from build123d import *

# Parameters (mm, degrees)
SKETCH1_W           = 127
SKETCH1_H           = 38.1
SKETCH1_R           = 15
BOSS_EXTRUDE1_DEPTH = 21
BOSS_EXTRUDE2_DEPTH = 6.35
SKETCH4_R           = 1.4
CUT_EXTRUDE2_DEPTH  = 6.35
CUT_EXTRUDE6_DEPTH  = 14.65
CUT_EXTRUDE7_DEPTH  = 73.600774789
SKETCH7_R           = 2.6035
CUT_EXTRUDE8_DEPTH  = 22.86
SKETCH8_W           = 31.75
SKETCH8_H           = 15.875
SKETCH8_R           = 2.6035
BOSS_EXTRUDE3_DEPTH = 9.652
CHAMFER1_SIZE       = 6.35
BOSS_EXTRUDE4_START = -9.652
SKETCH9_W           = 26.681402361
SKETCH9_H           = 11.886393241
SKETCH9_R           = 2.6035
SKETCH9_W_2         = 26.993648234
BOSS_EXTRUDE4_DEPTH = 9.652


with BuildPart() as part:
    # Sketch1 → Boss-Extrude1 (new body)
    with BuildSketch(Plane.XY):
        Rectangle(SKETCH1_W, SKETCH1_H)
        Circle(SKETCH1_R, mode=Mode.SUBTRACT)
    extrude(amount=-BOSS_EXTRUDE1_DEPTH)

    # Sketch3 → Boss-Extrude2 (add)
    with BuildSketch(Plane(origin=(0, 0, -21), x_dir=(-1, 0, 0), z_dir=(0, 0, -1))):
        with BuildLine():
            Line((12.743745366, -19.05), (-12.743745366, -19.05))
            ThreePointArc((-12.743745366, -19.05), (-9.084403439, -28.194328353), (1.02e-07, -32))
            ThreePointArc((1.02e-07, -32), (9.08440351, -28.194328281), (12.743745366, -19.05))
        make_face()
    boss_extrude2 = extrude(amount=-BOSS_EXTRUDE2_DEPTH)

    # Sketch4 → Cut-Extrude2 (cut)
    with BuildSketch(Plane.XY.offset(-14.65)):
        with Locations((0, -27)):
            Circle(SKETCH4_R)
    cut_extrude2 = extrude(amount=-CUT_EXTRUDE2_DEPTH, mode=Mode.SUBTRACT)

    # Mirror1: Boss-Extrude2, Cut-Extrude2 across plane
    add(boss_extrude2.mirror(Plane.ZX))
    add(cut_extrude2.mirror(Plane.ZX), mode=Mode.SUBTRACT)

    # Sketch5 → Cut-Extrude6 (cut)
    with BuildSketch(Plane.XY):
        with BuildLine():
            Line((-31.75, -4.826), (-63.5, -4.826))
            Line((-63.5, -4.826), (-63.5, -19.05))
            Line((-63.5, -19.05), (63.5, -19.05))
            Line((63.5, -19.05), (63.5, -4.826))
            Line((63.5, -4.826), (31.75, -4.826))
            ThreePointArc((31.75, -4.826), (0, -17.39350594), (-31.75, -4.826))
        make_face()
        with BuildLine():
            Line((-63.5, 19.05), (-63.5, 4.826))
            Line((-63.5, 4.826), (-31.75, 4.826))
            ThreePointArc((-31.75, 4.826), (0, 17.39350594), (31.75, 4.826))
            Line((31.75, 4.826), (63.5, 4.826))
            Line((63.5, 4.826), (63.5, 19.05))
            Line((63.5, 19.05), (-63.5, 19.05))
        make_face()
    extrude(amount=-CUT_EXTRUDE6_DEPTH, mode=Mode.SUBTRACT)

    # Sketch6 → Cut-Extrude7 (cut, through all)
    with BuildSketch(Plane.XY.offset(-14.65)):
        with BuildLine():
            Line((27.206467014, -8.577889412), (12.743745366, -19.05))
            Line((12.743745366, -19.05), (63.5, -19.05))
            Line((63.5, -19.05), (63.5, -4.826))
            Line((63.5, -4.826), (31.75, -4.826))
            ThreePointArc((31.75, -4.826), (29.537864162, -6.774157348), (27.206467014, -8.577889412))
        make_face()
        with BuildLine():
            Line((-63.5, -19.05), (-12.743745366, -19.05))
            Line((-12.743745366, -19.05), (-27.206467014, -8.577889412))
            ThreePointArc((-27.206467014, -8.577889412), (-29.537864162, -6.774157348), (-31.75, -4.826))
            Line((-31.75, -4.826), (-63.5, -4.826))
            Line((-63.5, -4.826), (-63.5, -19.05))
        make_face()
        with BuildLine():
            Line((-27.206467014, 8.577889412), (-12.743745366, 19.05))
            Line((-12.743745366, 19.05), (-63.5, 19.05))
            Line((-63.5, 19.05), (-63.5, 4.826))
            Line((-63.5, 4.826), (-31.75, 4.826))
            ThreePointArc((-31.75, 4.826), (-29.537864162, 6.774157348), (-27.206467014, 8.577889412))
        make_face()
        with BuildLine():
            Line((63.5, 19.05), (12.743745366, 19.05))
            Line((12.743745366, 19.05), (27.206467014, 8.577889412))
            ThreePointArc((27.206467014, 8.577889412), (29.537864162, 6.774157348), (31.75, 4.826))
            Line((31.75, 4.826), (63.5, 4.826))
            Line((63.5, 4.826), (63.5, 19.05))
        make_face()
    extrude(amount=-CUT_EXTRUDE7_DEPTH, mode=Mode.SUBTRACT)

    # Sketch7 → Cut-Extrude8 (cut)
    with BuildSketch(Plane(origin=(0, 4.826, 0), x_dir=(1, 0, 0), z_dir=(0, 1, 0))):
        with Locations(Location((-57.785, 10.5, 0), (0, 0, 270))):
            Circle(SKETCH7_R)
        with Locations(Location((-37.465, 10.5, 0), (0, 0, 270))):
            Circle(SKETCH7_R)
        with Locations(Location((37.465, 10.5, 0), (0, 0, 270))):
            Circle(SKETCH7_R)
        with Locations(Location((57.785, 10.5, 0), (0, 0, 270))):
            Circle(SKETCH7_R)
    extrude(amount=-CUT_EXTRUDE8_DEPTH, mode=Mode.SUBTRACT)

    # Sketch8 → Boss-Extrude3 (add)
    # profile 1 of 4: a face of its own
    with BuildSketch(Plane.XZ.offset(4.826)):
        Polygon((63.5, 0), (31.75, 0), (28.950809181, 15.875), (60.700809181, 15.875), align=None)
    # profile 2 of 4: a face of its own
    with BuildSketch(Plane.XZ.offset(4.826)):
        with Locations((44.825809181, 23.8125)):
            Rectangle(SKETCH8_W, SKETCH8_H)
        with Locations(Location((34.665809181, 23.8125, 0), (0, 0, 270))):
            Circle(SKETCH8_R, mode=Mode.SUBTRACT)
        with Locations(Location((54.985809181, 23.8125, 0), (0, 0, 270))):
            Circle(SKETCH8_R, mode=Mode.SUBTRACT)
    # profile 3 of 4: a face of its own
    with BuildSketch(Plane.XZ.offset(4.826)):
        with Locations((-44.825809181, 23.8125)):
            Rectangle(SKETCH8_W, SKETCH8_H)
        with Locations(Location((-34.665809181, 23.8125, 0), (0, 0, 270))):
            Circle(SKETCH8_R, mode=Mode.SUBTRACT)
        with Locations(Location((-54.985809181, 23.8125, 0), (0, 0, 270))):
            Circle(SKETCH8_R, mode=Mode.SUBTRACT)
    # profile 4 of 4: a face of its own
    with BuildSketch(Plane.XZ.offset(4.826)):
        Polygon((-60.700809181, 15.875), (-28.950809181, 15.875), (-31.75, 0), (-63.5, 0), align=None)
    extrude(amount=-BOSS_EXTRUDE3_DEPTH)

    # Chamfer1
    chamfer1_edges = [part.edges().sort_by_distance(p)[0] for p in [
        (28.950809181, 0, 31.75),
        (-28.950809181, 0, 31.75),
    ]]
    chamfer(chamfer1_edges, length=CHAMFER1_SIZE)

    # Sketch9 → Boss-Extrude4 (add)
    # profile 1 of 4: a face of its own
    with BuildSketch(Plane.XZ.offset(4.826).offset(BOSS_EXTRUDE4_START)):
        with Locations((-47.360108001, -9.539491199)):
            Rectangle(SKETCH9_W, SKETCH9_H)
        with Locations((-57.785, -10.5)):
            Circle(SKETCH9_R, mode=Mode.SUBTRACT)
        with Locations((-37.465, -10.5)):
            Circle(SKETCH9_R, mode=Mode.SUBTRACT)
    # profile 2 of 4: a face of its own
    with BuildSketch(Plane.XZ.offset(4.826).offset(BOSS_EXTRUDE4_START)):
        with Locations((-57.785, -10.5)):
            Circle(SKETCH9_R)
    # profile 3 of 4: a face of its own
    with BuildSketch(Plane.XZ.offset(4.826).offset(BOSS_EXTRUDE4_START)):
        with Locations((-37.465, -10.5)):
            Circle(SKETCH9_R)
    # profile 4 of 4: a face of its own
    with BuildSketch(Plane.XZ.offset(4.826).offset(BOSS_EXTRUDE4_START)):
        with Locations((47.713125711, -9.539491199)):
            Rectangle(SKETCH9_W_2, SKETCH9_H)
    extrude(amount=BOSS_EXTRUDE4_DEPTH)


solid = part.part
The model under review builds one solid part; all positions refer to its coordinate system, in mm. A direction names the side the tool comes from. Coordinates: 2 decimals unless noted, no trailing zeros. Write each loop counter-clockwise with the first axis right and the second up, starting at its lowest first coordinate (ties: lowest second). Pieces come first, ordered by that corner, then holes. Notation, with made-up numbers: (68.25, 77) - (97.25, 77) arc R24 ccw to (97.25, 115) - close; hole circle Ø4 at (-7, 42). An arc over 180 degrees is marked (long way). Answer as a JSON object with one key per item and string values. Group by question number.
1. Add section C-C (x = -9). Give the boundary of the cut face in (y, z), plus the area to 3 significant figures.
2. Clearance check with flat-ended pins moving along their axes: pin 1 Ø6 at (x, z) = (41.5, -13) entering from -Y; pin 2 Ø5 at (y, z) = (-1.5, 21.5) entering from +X; pin 3 Ø4 at (x, z) = (-54.99, 23.81) entering from -Y; pin 4 Ø5 at (y, z) = (1.5, 23) entering from -X. State where each tip first meets the part, or that it passes through.
3. Add section A-A (z = -9.5). Give the boundary of the cut face in (x, y).
4. Mouldability with a two-part tool opening along X and no side actions: class faces 1 (the face through (-46, -4.826, 6)), 2 (the face through (-60.701, 0, 24)), 3 (the face through (-32.17, -0.07, 28.62)) as pulls with the +X half, pulls with the -X half, needs draft (parallel to the pull), parting line crosses it, or undercut.
5. To check wall thickness, follow probe 1 along Y at (x, z) = (0, -15.5); probe 2 along Y at (x, z) = (0, -10); probe 3 along X at (y, z) = (-0.5, 22.5). State the ranges of each line that lie inside material, in increasing order.
6. Machinability: for faces 4 (the face through (20.08, -13.74, -17.78)), 5 (the face through (28.951, 0, 21)), which of the approach directions +Z, -Z, +X, -X, +Y, -Y give a long, thin tool a straight path to every point of the face, cutting with its end or side? Answer none if there is none.
7. Add section B-B (y = 1.5). Give the number of separate pieces and of enclosed holes in the cut face, plus the area to 3 significant figures.
8. Add section D-D (y = -12.5). Give the boundary of the cut face in (x, z).
Findings:
{
 "1": {"outline": "(-28.28, -21) - (-12, -21) - (-12, 0) - (-16.51, 0) - (-16.51, -14.65) - (-28.28, -14.65) - close; (12, -21) - (28.28, -21) - (28.28, -14.65) - (16.51, -14.65) - (16.51, 0) - (12, 0) - close", "area": "339 mm²"},
 "2": {"pin 1": "y = -4.83", "pin 2": "x = 60.7", "pin 3": "through", "pin 4": "x = -60.7"},
 "3": {"outline": "(-63.5, -4.83) - (-31.75, -4.83) arc R46.39 ccw to (31.75, -4.83) - (63.5, -4.83) - (63.5, 4.83) - (31.75, 4.83) arc R46.39 ccw to (-31.75, 4.83) - (-63.5, 4.83) - close; hole circle Ø30 at (0, 0)"},
 "4": {"face 1": "needs draft", "face 2": "pulls with the -X half", "face 3": "undercut"},
 "5": {"probe 1": "-32 to -28.4, -25.6 to -15, 15 to 25.6, 28.4 to 32", "probe 2": "-17.39 to -15, 15 to 17.39", "probe 3": "-60.7 to -57.23, -52.74 to -36.91, -32.42 to -28.95, 28.95 to 32.42, 36.91 to 52.74, 57.23 to 60.7"},
 "6": {"face 4": "+Z, -Z, +X, -Y", "face 5": "+Z, +Y, -Y"},
 "7": {"separate pieces": "2", "enclosed holes": "4", "area": "3,930 mm²"},
 "8": {"outline": "(-21.79, -21) - (-8.29, -21) - (-8.29, 0) - (-20.74, 0) - (-20.74, -14.65) - (-21.79, -14.65) - close; (8.29, -21) - (21.79, -21) - (21.79, -14.65) - (20.74, -14.65) - (20.74, 0) - (8.29, 0) - close"}
}
